from build123d import *

# Parameters (mm, degrees)
SKETCH1_R           = 5
BOSS_EXTRUDE1_DEPTH = 110
SKETCH2_R           = 8
BOSS_EXTRUDE2_DEPTH = 10
CHAMFER1_SIZE       = 0.5


with BuildPart() as part:
    # Sketch1 → Boss-Extrude1 (new body)
    with BuildSketch(Plane.XY):
        Circle(SKETCH1_R)
    extrude(amount=BOSS_EXTRUDE1_DEPTH)

    # Sketch2 → Boss-Extrude2 (add)
    with BuildSketch(Plane(origin=(0, 0, 0), x_dir=(-1, 0, 0), z_dir=(0, 0, -1))):
        Circle(SKETCH2_R)
    extrude(amount=BOSS_EXTRUDE2_DEPTH)

    # Chamfer1
    chamfer1_edges = [part.edges().sort_by_distance(p)[0] for p in [
        (-5, 0, 110),
        (8, 0, 0),
        (8, 0, -10),
    ]]
    chamfer(chamfer1_edges, length=CHAMFER1_SIZE)


solid = part.part
Source: CAD feature listing. Evaluate the final solid. Frame: model axes, mm. A direction names the side the tool comes from. Give positions to 0.01 mm unless a question says otherwise; leave off trailing zeros. Write each loop counter-clockwise with the first axis right and the second up, starting at its lowest first coordinate (ties: lowest second). Pieces come first, ordered by that corner, then holes. Notation, with made-up numbers: (19.5, 55) -> (36.5, 55) arc R12 ccw to (36.5, 65) -> close; hole circle Ø10 at (-24.5, -38.5). An arc over 180 degrees is marked (long way). Write item = value, one per line.
Q1. Cut plane A-A on y = 0. Return loops of the section in (x, z), then the cut area to 3 significant figures.
Here are the results:
outline = (-8, -9.5) -> (-7.5, -10) -> (7.5, -10) -> (8, -9.5) -> (8, -0.5) -> (7.5, 0) -> (5, 0) -> (5, 109.5) -> (4.5, 110) -> (-4.5, 110) -> (-5, 109.5) -> (-5, 0) -> (-7.5, 0) -> (-8, -0.5) -> close
area = 1,260 mm²
Q2. Line query: line 1 (Z direction, x = 5.5, y = -3.75); line 2 (X direction, y = 3, z = 42); line 3 (X direction, y = -3.75, z = -4.5). Output: solid intervals per line, ascending. Write a range as from..to.
Here are the results:
line_1 = -10..0
line_2 = -4..4
line_3 = -7.07..7.07
Q3. Cut plane C-C on z = 17.5. Return loops of the section in (x, y).
Here are the results:
outline = circle Ø10 at (0, 0)
Q4. First-contact query: pin 1 (1.5 mm diameter, centred on y = -4.5, z = 16, fed in from -X); pin 2 (5 mm diameter, centred on x = 0, z = 16.5, fed in from -Y); pin 3 (3 mm diameter, centred on y = 5, z = 37.5, fed in from +X). Flat tips, straight axial feed; report the tip coordinate or a pass-through.
Here are the results:
pin_1 = -3.31
pin_2 = -5
pin_3 = 3.57
Q5. Reachability of faces 1 (the face through (0, 0, -10)), 2 (the face through (-1.08, -4.88, 53.98)) from +Z, -Z, +X, -X, +Y, -Y: full face, straight path, thin tool, end or side. Return the list, or none.
Here are the results:
face_1 = -Z, +X, -X, +Y, -Y
face_2 = +Z
